For this review, take the finished solid that the model builds, in its own axes (mm). A direction names the side the tool comes from. Coordinates: 2 decimals unless noted, no trailing zeros. Loops run counter-clockwise (first coordinate to the right, second up) from the corner with the lowest first, then second, coordinate; pieces in that order, holes last. Notation, with made-up numbers: (55.25, 53.5) -> (61.25, 53.5) arc R14 cw to (61.25, 67.5) -> close; hole circle Ø1 at (23.25, 8.25). An arc over 180 degrees is marked (long way). Answer in a Markdown table with one row per item.
from build123d import *

# Parameters (mm, degrees)
HORIZONTAL_ARM_PROFILE_R    = 9
HORIZONTAL_ARM_7MM_DEPTH    = 7
VERTICAL_ARM_PROFILE_R      = 9
VERTICAL_ARM_7MM_DEPTH      = 7
BEND_FILLET_R5_R            = 5
HORIZONTAL_ARM_FILLET_R14_R = 14
BEND_FILLET_R7_R            = 7


with BuildPart() as part:
    # Horizontal Arm Profile → Horizontal Arm 7mm (new body)
    with BuildSketch(Plane(origin=(0, 0, 0), x_dir=(1, 0, 0), z_dir=(0, 1, 0))):
        with BuildLine():
            Line((-17.022044531, 10.5), (-85, 10.5))
            Line((-85, 10.5), (-85, -10.5))
            Line((-85, -10.5), (-17.022044531, -10.5))
            ThreePointArc((-17.022044531, -10.5), (20, 0), (-17.022044531, 10.5))
        make_face()
        with Locations(Location((0, 0, 0), (0, 0, 270))):
            Circle(HORIZONTAL_ARM_PROFILE_R, mode=Mode.SUBTRACT)
    extrude(amount=-HORIZONTAL_ARM_7MM_DEPTH)

    # Vertical Arm Profile → Vertical Arm 7mm (add)
    with BuildSketch(Plane(origin=(-85, 0, 0), x_dir=(0, 0, -1), z_dir=(1, 0, 0))):
        with BuildLine():
            Line((-10.5, 0), (-10.5, -37.977955469))
            ThreePointArc((-10.5, -37.977955469), (0, -75), (10.5, -37.977955469))
            Line((10.5, -37.977955469), (10.5, 0))
            Line((10.5, 0), (-10.5, 0))
        make_face()
        with Locations((0, -55)):
            Circle(VERTICAL_ARM_PROFILE_R, mode=Mode.SUBTRACT)
    extrude(amount=VERTICAL_ARM_7MM_DEPTH)

    # Bend Fillet R5
    bend_fillet_r5_edges = [part.edges().sort_by_distance(p)[0] for p in [
        (-81.5, -37.977955469, -10.5),
        (-81.5, -37.977955469, 10.5),
        (-17.022044531, -3.5, 10.5),
        (-17.022044531, -3.5, -10.5),
    ]]
    fillet(bend_fillet_r5_edges, radius=BEND_FILLET_R5_R)

    # Horizontal Arm Fillet R14
    horizontal_arm_fillet_r14_edges = [part.edges().sort_by_distance(p)[0] for p in [
        (-85, 0, 0),
    ]]
    fillet(horizontal_arm_fillet_r14_edges, radius=HORIZONTAL_ARM_FILLET_R14_R)

    # Bend Fillet R7
    bend_fillet_r7_edges = [part.edges().sort_by_distance(p)[0] for p in [
        (-78, -7, 0),
    ]]
    fillet(bend_fillet_r7_edges, radius=BEND_FILLET_R7_R)


solid = part.part
Item 1: Take a section at A-A, the plane z = 0. State the section outline as (x, y) points.
Worked answers:
| item | result |
|---|---|
| outline | (-85, -75) -> (-78, -75) -> (-78, -64) -> (-85, -64) -> close; (-85, -46) -> (-78, -46) -> (-78, -14) arc R7 cw to (-71, -7) -> (-9, -7) -> (-9, 0) -> (-71, 0) arc R14 ccw to (-85, -14) -> close; (9, -7) -> (20, -7) -> (20, 0) -> (9, 0) -> close |
Item 2: Take a section at C-C, the plane y = -59. State the section outline as (x, z) points.
Worked answers:
| item | result |
|---|---|
| outline | (-85, -19.6) -> (-78, -19.6) -> (-78, -8.06) -> (-85, -8.06) -> close; (-85, 8.06) -> (-78, 8.06) -> (-78, 19.6) -> (-85, 19.6) -> close |
Item 3: Insertion check: pin 1 (12 mm diameter, centred on x = -3.5, z = -11, fed in from -Y); pin 2 (1 mm diameter, centred on y = -23.5, z = -4, fed in from +X); pin 3 (17.5 mm diameter, centred on x = -36, y = -14.5, fed in from -Z). Each pin has a flat end and moves straight along its axis. Give the tip position at first contact, or say it passes through.
Worked answers:
| item | result |
|---|---|
| pin 1 | y = -7 |
| pin 2 | x = -78 |
| pin 3 | z = -10.5 |
Item 4: For faces 1 (the flat face through (-62, -6, -10.5)), 2 (the cylindrical face through (-81.45, -37.54, 10.99)), 3 (the flat face through (-78, -44, 0)), list the 3-axis set-ups (+Z, -Z, +X, -X, +Y, -Y) from which the entire face can be reached by the end or side of a thin tool; tool diameter is ignored.
Worked answers:
| item | result |
|---|---|
| face 1 | -Z, -X, +Y |
| face 2 | +Z, +X, -X, +Y |
| face 3 | +Z, -Z, +X, -Y |
Item 5: Take a section at B-B, the plane x = 0. State the section outline as (y, z) points, and give its area (3 significant figures).
Worked answers:
| item | result |
|---|---|
| outline | (-7, -20) -> (0, -20) -> (0, -9) -> (-7, -9) -> close; (-7, 9) -> (0, 9) -> (0, 20) -> (-7, 20) -> close |
| area | 154 mm² |
Item 6: Take a section at D-D, the plane x = -63. State the section outline as (y, z) points.
Worked answers:
| item | result |
|---|---|
| outline | (-7, -10.5) -> (0, -10.5) -> (0, 10.5) -> (-7, 10.5) -> close |
Item 7: For L1, parallel to Y at x = -37.5, z = -5; L2, parallel to Z at x = -21, y = -6; L3, parallel to Y at x = -81, z = 0, list the stretches that pass through material, from the lowest coordinate up.
Worked answers:
| item | result |
|---|---|
| L1 | -7 to 0 |
| L2 | -10.5 to 10.5 |
| L3 | -75 to -64, -46 to -4.2 |
Item 8: The part is to be moulded in two halves that separate along Z. For faces 4 (the flat face through (-60, -6, 10.5)), 5 (the cylindrical face through (-17.46, -3.55, -10.99)), 6 (the cylindrical face through (-75.9, -9, -0.1)), 7 (the cylindrical face through (2.703, -3.451, 8.584)), say which applies: +Z half, -Z half, draft (parallel to the pull), parting line (faces both ways), or undercut.
Worked answers:
| item | result |
|---|---|
| face 4 | +Z half |
| face 5 | -Z half |
| face 6 | draft |
| face 7 | undercut |
